The figure shows three views and two pictorial views of one solid part (mm, origin at its lowest corner). Answer the questions. A direction names the side the tool comes from. Give positions to 0.01 mm unless a question says otherwise; leave off trailing zeros. Write each loop counter-clockwise with the first axis right and the second up, starting at its lowest first coordinate (ties: lowest second). Pieces come first, ordered by that corner, then holes. Notation, with made-up numbers: M -36,-16.75 L -15,-16.75 A15 cw -15,11.25 Z; hole C -21.75,38 d3. An arc over 180 degrees is marked long. Return JSON: item names as keys, results as strings.
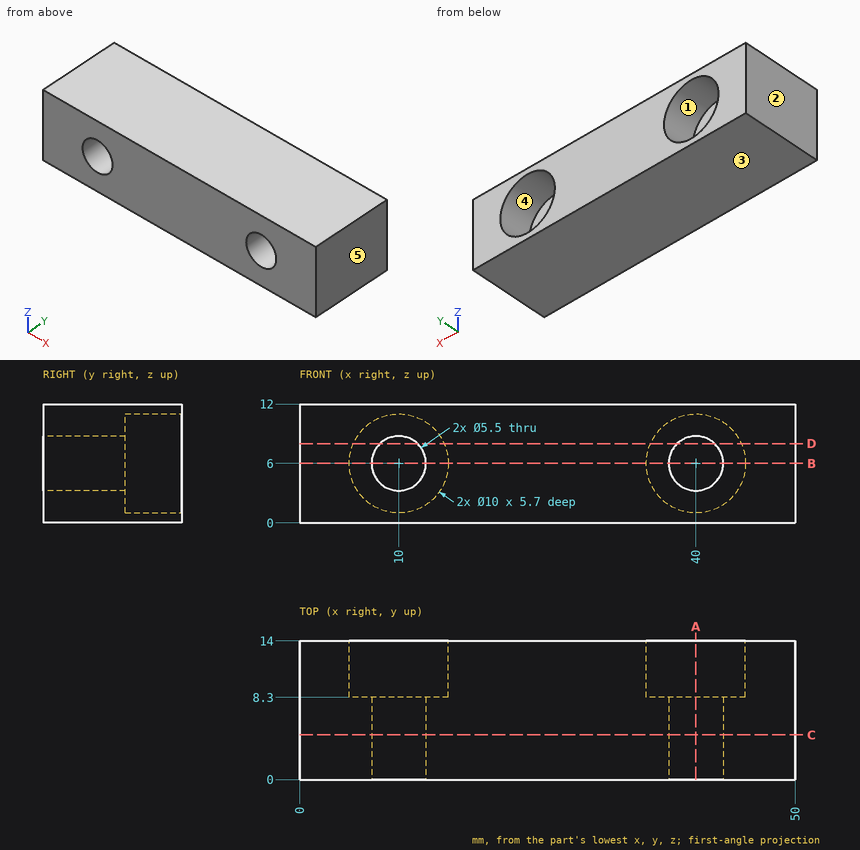
Item 1: Which of the six approach directions +Z, -Z, +X, -X, +Y, -Y give full straight-line access (tool end or side, diameter ignored) to the marked faces 1 and 2?
Geometry results:
{"face 1": "+Y", "face 2": "+Z, -Z, -X, +Y, -Y"}
Item 2: A cutting plane is placed at C-C, the plane y = 4.5. Write down the section's boundary in (x, z).
Geometry results:
{"outline": "M 0,0 L 50,0 L 50,12 L 0,12 Z; hole C 10,6 d5.5; hole C 40,6 d5.5"}
Item 3: A cutting plane is placed at A-A, the plane x = 40. Write down the section's boundary in (y, z), plus the area to 4 significant figures.
Geometry results:
{"outline": "M 0,0 L 14,0 L 14,1 L 8.3,1 L 8.3,3.25 L 0,3.25 Z; M 0,8.75 L 8.3,8.75 L 8.3,11 L 14,11 L 14,12 L 0,12 Z", "area": "65.35 mm2"}
Item 4: A cutting plane is placed at B-B, the plane z = 6. Write down the section's boundary in (x, y).
Geometry results:
{"outline": "M 0,0 L 7.25,0 L 7.25,8.3 L 5,8.3 L 5,14 L 0,14 Z; M 12.75,0 L 37.25,0 L 37.25,8.3 L 35,8.3 L 35,14 L 15,14 L 15,8.3 L 12.75,8.3 Z; M 42.75,0 L 50,0 L 50,14 L 45,14 L 45,8.3 L 42.75,8.3 Z"}
Item 5: A cutting plane is placed at D-D, the plane z = 8. Write down the section's boundary in (x, y).
Geometry results:
{"outline": "M 0,0 L 8.11,0 L 8.11,8.3 L 5.42,8.3 L 5.42,14 L 0,14 Z; M 11.89,0 L 38.11,0 L 38.11,8.3 L 35.42,8.3 L 35.42,14 L 14.58,14 L 14.58,8.3 L 11.89,8.3 Z; M 41.89,0 L 50,0 L 50,14 L 44.58,14 L 44.58,8.3 L 41.89,8.3 Z"}
Item 6: Given pin 1 Ø3 at (x, z) = (28, 4.5) entering from -Y; pin 2 Ø3.5 at (x, z) = (10, 6) entering from +Y, each flat-ended and moving along its own axis, determine where each tip first touches the part or whether it passes through.
Geometry results:
{"pin 1": "stops at y = 0", "pin 2": "passes through"}
Item 7: Find the intervals of material crossed by line 1 (Z direction, x = 40, y = 4); line 2 (X direction, y = 2.5, z = 4); line 3 (Y direction, x = 6.5, z = 8), in increasing order.
Geometry results:
{"line 1": "z = 0 to 3.25, 8.75 to 12", "line 2": "x = 0 to 8.11, 11.89 to 38.11, 41.89 to 50", "line 3": "y = 0 to 8.3"}
Item 8: Determine the mould class of the marked faces 3, 4 and 5 for opening direction Z: +Z half, -Z half, draft (parallel to the pull), parting line (faces both ways), or undercut.
Geometry results:
{"face 3": "-Z half", "face 4": "undercut", "face 5": "draft"}
